Read the model definition and answer for the solid it produces. Units are mm, in the model's axes. Face numbers are marked on the shaded views. A direction names the side the tool comes from. Give positions to 0.01 mm unless a question says otherwise; leave off trailing zeros. Order: outer loops, then holes, each group sorted by start corner. A loop starts at its lowest first (then second) coordinate and runs counter-clockwise, first axis right, second up. Notation, with made-up numbers: (35, 43) -> (71, 43) arc R18 cw to (71, 76) -> close; hole circle Ø6 at (74.5, -29). An arc over 180 degrees is marked (long way). Use one line per item in the form item = value.
```python
from build123d import *

# Parameters (mm, degrees)
BOSS_EXTRUDE1_DEPTH            = 20
CUT_EXTRUDE1_REACH             = 326.283
SKETCH2_W                      = 10
SKETCH2_H                      = 33.118542384
CUT_EXTRUDE2_DEPTH             = 329.583692554
F_15_0_15_DIAMETER_HOLE1_D     = 15
F_15_0_15_DIAMETER_HOLE1_DEPTH = 5
F_15_0_15_DIAMETER_HOLE2_D     = 15
F_15_0_15_DIAMETER_HOLE3_D     = 15
FILLET1_R                      = 5
FILLET2_R                      = 15
CUT_EXTRUDE3_DEPTH             = 20
SCALE1_SCALE                   = 0.3


with BuildPart() as part:
    # Sketch1 → Boss-Extrude1 (new body)
    with BuildSketch(Plane.XY.offset(20)):
        with BuildLine():
            Line((-35.601097413, 326.0365085), (-35.601097413, 70.746699079))
            Line((-35.601097413, 70.746699079), (-14.395848526, 12.48575659))
            ThreePointArc((-14.395848526, 12.48575659), (4.829842935, 3.520669429), (13.794930097, 22.74636089))
            Line((13.794930097, 22.74636089), (-5.601097413, 76.0365085))
            Line((-5.601097413, 76.0365085), (-5.601097413, 326.0365085))
            Line((-5.601097413, 326.0365085), (-35.601097413, 326.0365085))
        make_face()
    extrude(amount=-BOSS_EXTRUDE1_DEPTH)

    # Sketch2 → Cut-Extrude1 (cut, up to next)
    with BuildSketch(Plane(origin=(19.491769294, 7.094423836, 0), x_dir=(0, 0, -1), z_dir=(0.9396926207859105, 0.3420201433256631, 0)), mode=Mode.PRIVATE) as cut_extrude1_sk1:
        with Locations((-10, 15.602274889)):
            Rectangle(SKETCH2_W, SKETCH2_H)
    cut_extrude1_tool1 = extrude(cut_extrude1_sk1.sketch, amount=-CUT_EXTRUDE1_REACH, mode=Mode.PRIVATE) & part.part
    add(cut_extrude1_tool1.solids().sort_by_distance((14.155477, 21.755766, 10))[0], mode=Mode.SUBTRACT)

    # Sketch3 → Cut-Extrude2 (cut, through all)
    with BuildSketch(Plane(origin=(0, 0, 0), x_dir=(-1, 0, 0), z_dir=(0, 0, -1))):
        with BuildLine():
            Line((35.601097413, 84.169572779), (35.601097413, 254.427504812))
            Line((35.601097413, 254.427504812), (25.601097413, 246.0365085))
            Line((25.601097413, 246.0365085), (25.601097413, 106.530252554))
            ThreePointArc((25.601097413, 106.530252554), (26.908033475, 100.406528198), (30.601097413, 95.349912667))
            ThreePointArc((30.601097413, 95.349912667), (34.29416135, 90.293297136), (35.601097413, 84.169572779))
        make_face()
    extrude(amount=-CUT_EXTRUDE2_DEPTH, mode=Mode.SUBTRACT)

    # Ø15.0 (15) Diameter Hole1
    with Locations(Plane.XY.offset(5)):
        with Locations((-0.300459215, 17.61605874)):
            Hole(F_15_0_15_DIAMETER_HOLE1_D / 2, depth=F_15_0_15_DIAMETER_HOLE1_DEPTH)

    # Ø15.0 (15) Diameter Hole2 (through all)
    with Locations(Plane(origin=(0, 0, 0), x_dir=(-1, 0, 0), z_dir=(0, 0, -1))):
        with Locations((21.505708101, 75.877001229)):
            Hole(F_15_0_15_DIAMETER_HOLE2_D / 2)

    # Ø15.0 (15) Diameter Hole3 (through all)
    with Locations(Plane(origin=(0, 0, 15), x_dir=(-1, 0, 0), z_dir=(0, 0, -1))):
        with Locations((0.300459215, 17.61605874)):
            Hole(F_15_0_15_DIAMETER_HOLE3_D / 2)

    # Fillet1
    fillet1_edges = [part.edges().sort_by_distance(p)[0] for p in [
        (8.491872693, 37.316391362, 10),
    ]]
    fillet(fillet1_edges, radius=FILLET1_R)

    # Fillet2
    fillet2_edges = [part.edges().sort_by_distance(p)[0] for p in [
        (-5.601097413, 326.0365085, 10),
        (-5.601097413, 76.0365085, 10),
        (-35.601097413, 70.746699079, 10),
        (-25.601097413, 246.0365085, 10),
    ]]
    fillet(fillet2_edges, radius=FILLET2_R)

    # Sketch10 → Cut-Extrude3 (cut)
    with BuildSketch(Plane.XY.offset(20)):
        Polygon((-35.601097413, 317.362498495), (-35.601097413, 321.974448946), (-35.601097413, 326.0365085), (-41.358567597, 326.0365085), (-41.358567597, 256.644428456), (-35.601097413, 256.644428456), (-35.601097413, 261.256378908), (-35.601097413, 265.318438462), (-35.601097413, 269.930388913), (-35.601097413, 273.992448467), (-35.601097413, 278.604398919), (-35.601097413, 282.666458473), (-35.601097413, 287.278408924), (-35.601097413, 291.340468478), (-35.601097413, 295.95241893), (-35.601097413, 300.014478484), (-35.601097413, 304.626428935), (-35.601097413, 308.688488489), (-35.601097413, 313.300438941), align=None)
        Polygon((-31.945953564, 310.813956834), (-35.601097413, 313.300438941), (-35.601097413, 308.688488489), align=None)
        Polygon((-31.945953564, 319.487966839), (-35.601097413, 321.974448946), (-35.601097413, 317.362498495), align=None)
        Polygon((-31.945953564, 302.139946828), (-35.601097413, 304.626428935), (-35.601097413, 300.014478484), align=None)
        Polygon((-31.945953564, 293.465936823), (-35.601097413, 295.95241893), (-35.601097413, 291.340468478), align=None)
        Polygon((-31.945953564, 284.791926817), (-35.601097413, 287.278408924), (-35.601097413, 282.666458473), align=None)
        Polygon((-35.601097413, 278.604398919), (-35.601097413, 273.992448467), (-31.945953564, 276.117916812), align=None)
        Polygon((-35.601097413, 269.930388913), (-35.601097413, 265.318438462), (-31.945953564, 267.443906806), align=None)
        Polygon((-35.601097413, 261.256378908), (-35.601097413, 256.644428456), (-31.945953564, 258.769896801), align=None)
    extrude(amount=-CUT_EXTRUDE3_DEPTH, mode=Mode.SUBTRACT)


with BuildPart() as part_1:
    # Scale1: scaled about (0, 0, 0)
    add(part.part.scale(SCALE1_SCALE))


solid = part_1.part
```
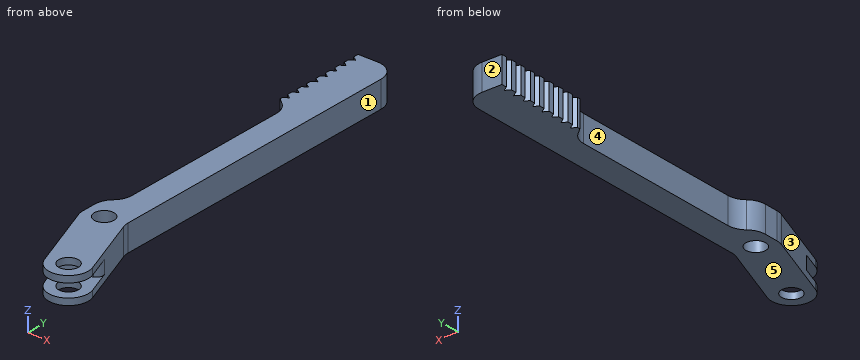
Item 1: The part is cut by section A-A on y = 69. Give the vertices of the cut face in (x, z), and give its area (3 significant figures).
Checks:
outline = (-7.68, 0) -> (-1.68, 0) -> (-1.68, 6) -> (-7.68, 6) -> close
area = 36.0 mm²
Item 2: Which of the six approach directions +Z, -Z, +X, -X, +Y, -Y give full straight-line access (tool end or side, diameter ignored) to the marked faces 1 and 2?
Checks:
face_1 = +Z, -Z, +X, +Y
face_2 = +Z, -Z, +X, -X, +Y
Item 3: Given pin 1 Ø2 at (x, y) = (1, 82.5) entering from +Z; pin 2 Ø1.8 at (y, z) = (43.5, 2.5) entering from -X; pin 3 Ø3 at (y, z) = (60, 4.5) entering from +X, each flat-ended and moving along its own axis, determine where each tip first touches the part or whether it passes through.
Checks:
pin_1 = through
pin_2 = -7.68
pin_3 = -1.68
Item 4: Straight lines are drawn through the part: L1, parallel to X at y = 51, z = 4.35; L2, parallel to X at y = 77, z = 2.05; L3, parallel to Y at x = -3.5, z = 4.8. For each, find the intervals that lie inside material, in ascending order. Write a range as from..to.
Checks:
L1 = -7.68..-1.68
L2 = -10.67..-1.68
L3 = 2.35..96.93
Item 5: The part is cut by section B-B on y = 17. Give the vertices of the cut face in (x, z).
Checks:
outline = (-9.14, 0) -> (0.43, 0) -> (0.43, 6) -> (-9.14, 6) -> close
Item 6: Determine the mould class of the marked faces 3, 4 and 5 for opening direction Y: +Y half, -Y half, draft (parallel to the pull), parting line (faces both ways), or undercut.
Checks:
face_3 = -Y half
face_4 = undercut
face_5 = draft
